```python
from build123d import *

# Parameters (mm, degrees)
SKETCH_1_W              = 60
SKETCH_1_H              = 30
EXTRUDE_1_DEPTH         = 90
SKETCH_2_W              = 60
SKETCH_2_H              = 30
EXTRUDE_2_DEPTH         = 20
HOLE_WIZARD_9_0_9_1_D   = 9
HOLE_WIZARD_M16_1_D     = 14
HOLE_WIZARD_M16_1_DEPTH = 38
HOLE_WIZARD_M16_1_TIP   = 4.206024333
CHAMFER_1_SIZE          = 5
CHAMFER_2_SIZE          = 5


with BuildPart() as part:
    # 草图1 → 凸台-拉伸1 (new body)
    with BuildSketch(Plane.XY):
        Rectangle(SKETCH_1_W, SKETCH_1_H)
    extrude(amount=EXTRUDE_1_DEPTH)

    # 草图2 → 凸台-拉伸2 (add)
    with BuildSketch(Plane(origin=(0, 15, 0), x_dir=(1, 0, 0), z_dir=(0, 1, 0))):
        with Locations((0, -75)):
            Rectangle(SKETCH_2_W, SKETCH_2_H)
    extrude(amount=EXTRUDE_2_DEPTH)

    # Ø9.0 (9) 直径孔1 (through all)
    with Locations(Plane(origin=(0, 15, 0), x_dir=(1, 0, 0), z_dir=(0, 1, 0))):
        with Locations((-15, -15), (15, -15), (-15, -40), (15, -40)):
            Hole(HOLE_WIZARD_9_0_9_1_D / 2)

    # M16 螺纹孔1
    with Locations(Plane.XY.offset(90)):
        with Locations((0, 14)):
            Hole(HOLE_WIZARD_M16_1_D / 2, depth=HOLE_WIZARD_M16_1_DEPTH)
            with Locations((0, 0, -(HOLE_WIZARD_M16_1_DEPTH + HOLE_WIZARD_M16_1_TIP / 2))):  # 118° drill point
                Cone(0, HOLE_WIZARD_M16_1_D / 2, HOLE_WIZARD_M16_1_TIP, mode=Mode.SUBTRACT)

    # 倒角1
    chamfer_1_edges = [part.edges().sort_by_distance(p)[0] for p in [
        (-30, 35, 75),
        (30, 35, 75),
        (-30, 0, 0),
        (30, 0, 0),
    ]]
    chamfer(chamfer_1_edges, length=CHAMFER_1_SIZE)

    # 倒角2
    chamfer_2_edges = [part.edges().sort_by_distance(p)[0] for p in [
        (0, -15, 90),
    ]]
    chamfer(chamfer_2_edges, length=CHAMFER_2_SIZE)


solid = part.part
```
Verification items for the finished model (mm, model axes). A direction names the side the tool comes from. Round coordinates to 2 decimals unless told otherwise and drop trailing zeros. Loops run counter-clockwise (first coordinate to the right, second up) from the corner with the lowest first, then second, coordinate; pieces in that order, holes last. Notation, with made-up numbers: (-22, 4.5) -> (10, 4.5) arc R25 cw to (10, 30.5) -> close; hole circle Ø10 at (75, 41.25). An arc over 180 degrees is marked (long way). Answer as a JSON object with one key per item and string values.
Q1. Section check A-A (z = 40). Record the boundary of the cut face in (x, y), then the cut area to 3 significant figures.
Data:
{"outline": "(-30, -15) -> (-19.5, -15) -> (-19.5, 15) -> (-30, 15) -> close; (-10.5, -15) -> (10.5, -15) -> (10.5, 15) -> (-10.5, 15) -> close; (19.5, -15) -> (30, -15) -> (30, 15) -> (19.5, 15) -> close", "area": "1,260 mm2"}
Q2. Section check B-B (x = -15). Record the boundary of the cut face in (y, z).
Data:
{"outline": "(-15, 0) -> (15, 0) -> (15, 10.5) -> (-15, 10.5) -> close; (-15, 19.5) -> (15, 19.5) -> (15, 35.5) -> (-15, 35.5) -> close; (-15, 44.5) -> (15, 44.5) -> (15, 60) -> (35, 60) -> (35, 90) -> (-10, 90) -> (-15, 85) -> close"}
Q3. Access from +Z, -Z, +X, -X, +Y, -Y to the whole of each face (thin tool, end or side, straight path). Record for faces 1 (the flat face through (-7, 12, 90)), 2 (the flat face through (0, 15, 30)), 3 (the cylindrical face through (1.517, 7.166, 70.734)).
Data:
{"face 1": "+Z, +X, -X, +Y, -Y", "face 2": "-Z, +X, -X, +Y", "face 3": "+Z"}
Q4. Scan lines: line 1 (Z direction, x = 15, y = -7); line 2 (X direction, y = -7, z = 40); line 3 (X direction, y = -7, z = 36). Record each from-to range of solid material in increasing order. Write a range as from..to.
Data:
{"line 1": "z = 0..10.5, 19.5..35.5, 44.5..90", "line 2": "x = -30..-19.5, -10.5..10.5, 19.5..30", "line 3": "x = -30..-17.06, -12.94..12.94, 17.06..30"}
Q5. Draft check along Z on faces 4 (the cylindrical face through (15.98, -0.21, 44.39)), 5 (the flat face through (0, 25, 60)), 6 (the flat face through (0, -13, 87)). Enter one of: pulls with the +Z half, pulls with the -Z half, needs draft (parallel to the pull), parting line crosses it, or undercut.
Data:
{"face 4": "undercut", "face 5": "pulls with the -Z half", "face 6": "pulls with the +Z half"}
Q6. Section check C-C (y = -7). Record the boundary of the cut face in (x, z).
Data:
{"outline": "(-30, 5) -> (-25, 0) -> (25, 0) -> (30, 5) -> (30, 90) -> (-30, 90) -> close; hole circle Ø9 at (-15, 15); hole circle Ø9 at (-15, 40); hole circle Ø9 at (15, 15); hole circle Ø9 at (15, 40)"}
Q7. Go/stop test with a flat-tipped pin: P1, Ø10, axis at x = 4.5, z = 45, coming from the +Y side. Record where the tip stops, or that it passes through.
Data:
{"P1": "stops at y = 15"}
Q8. Section check D-D (z = 79.5). Record the boundary of the cut face in (x, y), then the cut area to 3 significant figures.
Data:
{"outline": "(-30, -15) -> (30, -15) -> (30, 30) -> (25, 35) -> (-25, 35) -> (-30, 30) -> close; hole circle Ø14 at (0, 14)", "area": "2,820 mm2"}
